Geometry: final body of the model. Coordinates: model frame, mm. Face numbers are marked on the shaded views. A direction names the side the tool comes from. Round coordinates to 2 decimals unless told otherwise and drop trailing zeros. Loops run counter-clockwise (first coordinate to the right, second up) from the corner with the lowest first, then second, coordinate; pieces in that order, holes last. Notation, with made-up numbers: (-26.5, 51) - (-1.5, 51) arc R21 ccw to (-1.5, 66) - close; hole circle Ø3 at (11, 79). An arc over 180 degrees is marked (long way). Return JSON: item names as keys, results as strings. Group by question number.
1. Draft query along Z for the marked faces 3, 4 and 5. Return one class per face: +Z half, -Z half, draft (parallel to the pull), parting line (faces both ways), or undercut.
2. Material intervals for probe 1 along Y at (x, z) = (31, -76); probe 2 along Y at (x, z) = (31.5, 76); probe 3 along Z at (x, y) = (33, -65), sorted ascending.
3. First-contact query: pin 1 Ø3 at (y, z) = (-104, -19.5) entering from +X. Flat tip, straight axial feed; report the tip coordinate or a pass-through.
4. Section B-B on x = 9. Return loops of the section in (y, z), and give its area (4 significant figures).
5. Section C-C on z = -5.5. Return loops of the section in (x, y), and give its area (3 significant figures).
6. Set-up query: the marked faces 1 and 2. Return all of +Z, -Z, +X, -X, +Y, -Y with unobstructed straight access to the full face (end or side cutting, diameter ignored); none if empty.
7. Section A-A on y = -259. Return loops of the section in (x, z).
from build123d import *

# Parameters (mm, degrees)
SKETCH_2_W            = 83
SKETCH_2_H            = 153
EXTRUDE_2_DEPTH       = 297.5
CHAMFER_1_SIZE        = 15
FILLET_1_R            = 10
SHELL_2_T             = -1.5
HOLE_WIZARD_5_0_5_1_D = 5
FILLET_2_R            = 2


with BuildPart() as part:
    # 草图2 → 凸台-拉伸2 (new body)
    with BuildSketch(Plane(origin=(0, 0, 0), x_dir=(1, 0, 0), z_dir=(0, 1, 0))):
        Rectangle(SKETCH_2_W, SKETCH_2_H)
    extrude(amount=-EXTRUDE_2_DEPTH)

    # 倒角1
    chamfer_1_edges = [part.edges().sort_by_distance(p)[0] for p in [
        (-41.5, -148.75, 76.5),
        (-41.5, -148.75, -76.5),
    ]]
    chamfer(chamfer_1_edges, length=CHAMFER_1_SIZE)

    # 圆角1
    fillet_1_edges = [part.edges().sort_by_distance(p)[0] for p in [
        (-26.5, -148.75, -76.5),
        (-41.5, -148.75, 61.5),
        (-41.5, -148.75, -61.5),
        (-26.5, -148.75, 76.5),
    ]]
    fillet(fillet_1_edges, radius=FILLET_1_R)

    # 抽壳2
    shell_2_openings = [part.faces().sort_by_distance(p)[0] for p in [
        (0.682002961, -297.5, 0),
        (0.682002961, 0, 0),
        (41.5, -148.75, 0),
    ]]
    offset(amount=SHELL_2_T, openings=shell_2_openings, kind=Kind.INTERSECTION)

    # Ø5.0 (5) 直径孔1 (through all)
    with Locations(Plane.XY.offset(76.5)):
        with Locations((31.5, -17.5), (31.5, -147.5), (31.5, -277.5)):
            Hole(HOLE_WIZARD_5_0_5_1_D / 2)

    # 圆角2
    fillet_2_edges = [part.edges().sort_by_distance(p)[0] for p in [
        (41.5, -297.5, 75.75),
        (41.5, 0, -75.75),
        (41.5, -297.5, -75.75),
        (41.5, 0, 75.75),
    ]]
    fillet(fillet_2_edges, radius=FILLET_2_R)


solid = part.part
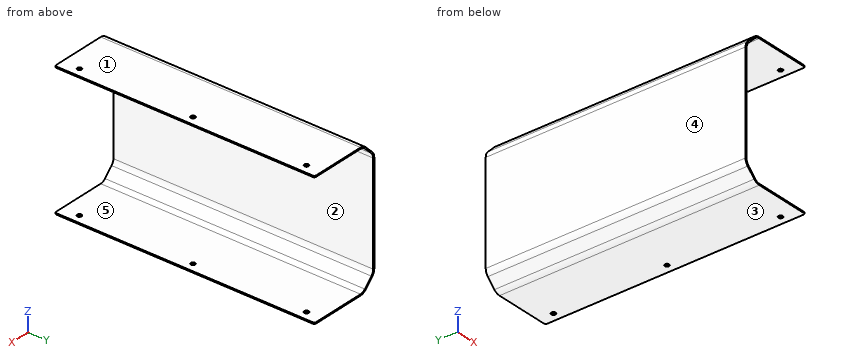
Taken from the geometry:
{
 "1": {"face 3": "-Z half", "face 4": "draft", "face 5": "undercut"},
 "2": {"probe 1": "-297.5 to -279.95, -275.05 to -149.95, -145.05 to -19.95, -15.05 to 0", "probe 2": "-297.5 to -280, -275 to -150, -145 to -20, -15 to 0", "probe 3": "-76.5 to -75, 75 to 76.5"},
 "3": {"pin 1": "x = -40"},
 "4": {"outline": "(-297.5, -76.5) - (0, -76.5) - (0, -75) - (-297.5, -75) - close; (-297.5, 75) - (0, 75) - (0, 76.5) - (-297.5, 76.5) - close", "area": "892.5 mm2"},
 "5": {"outline": "(-41.5, -297.5) - (-40, -297.5) - (-40, 0) - (-41.5, 0) - close", "area": "446 mm2"},
 "6": {"face 1": "+Z, +X, -X, +Y, -Y", "face 2": "+X, +Y, -Y"},
 "7": {"outline": "(-41.5, -57.36) arc R10 ccw to (-38.57, -64.43) - (-29.43, -73.57) arc R10 ccw to (-22.36, -76.5) - (41.5, -76.5) - (41.5, -75) - (-22.36, -75) arc R8.5 cw to (-28.37, -72.51) - (-37.51, -63.37) arc R8.5 cw to (-40, -57.36) - (-40, 57.36) arc R8.5 cw to (-37.51, 63.37) - (-28.37, 72.51) arc R8.5 cw to (-22.36, 75) - (41.5, 75) - (41.5, 76.5) - (-22.36, 76.5) arc R10 ccw to (-29.43, 73.57) - (-38.57, 64.43) arc R10 ccw to (-41.5, 57.36) - close"}
}
